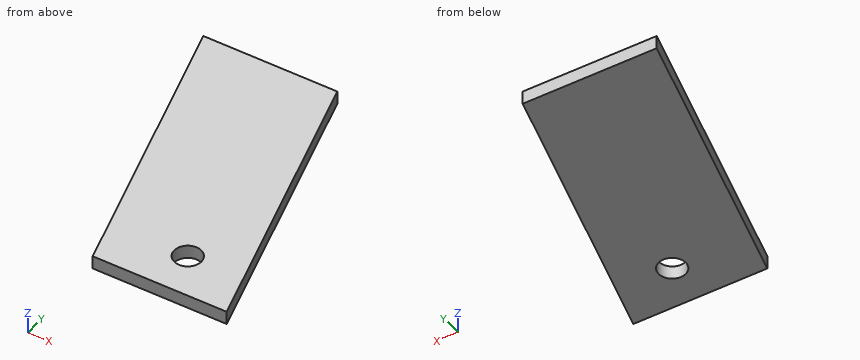
```python
from build123d import *

# Parameters (mm, degrees)
EXTRUDE_1_DEPTH     = 3
SKETCH_2_R          = 6.1
CUT_EXTRUDE_1_DEPTH = 15


with BuildPart() as part:
    # 草图1 → 凸台-拉伸1 (new, symmetric)
    with BuildSketch(Plane.XY):
        Polygon((-30, -36), (30, -36), (65, -167), (5, -167), align=None)
    extrude(amount=EXTRUDE_1_DEPTH, both=True)

    # 草图2 → 切除-拉伸1 (cut, symmetric)
    with BuildSketch(Plane.XY):
        with Locations(Location((35, -147.5, 0), (0, 0, 180))):
            Circle(SKETCH_2_R)
    extrude(amount=CUT_EXTRUDE_1_DEPTH, both=True, mode=Mode.SUBTRACT)


solid = part.part
```
The listing builds one solid part. Answer for the finished solid, in the listing's coordinates (mm). Give positions to 0.01 mm unless a question says otherwise; leave off trailing zeros. Order: outer loops, then holes, each group sorted by start corner. A loop starts at its lowest first (then second) coordinate and runs counter-clockwise, first axis right, second up.
1) Find section B-B on x = 35. Write down the section's boundary in (y, z).
Reported:
outline: (-167, -3) - (-153.6, -3) - (-153.6, 3) - (-167, 3) - close; (-141.4, -3) - (-54.71, -3) - (-54.71, 3) - (-141.4, 3) - close
2) Find section A-A on z = -0.6. Write down the section's boundary in (x, y), then the cut area to 3 significant figures.
Reported:
outline: (-30, -36) - (5, -167) - (65, -167) - (30, -36) - close; hole circle Ø12.2 at (35, -147.5)
area: 7,740 mm2
3) Consider line 1 along X through (y, z) = (-147.5, -0.4); line 2 along X through (y, z) = (-148.5, 1.55); line 3 along X through (y, z) = (-68.5, -1.55). Determine where each line is inside the solid, lowest interval first.
Reported:
line 1: x = -0.21 to 28.9, 41.1 to 59.79
line 2: x = 0.06 to 28.98, 41.02 to 60.06
line 3: x = -21.32 to 38.68
4) Given P1, Ø2, axis at y = -122, z = 0.5, coming from the +X side, flat-ended and moving along its own axis, determine where the tip first touches the part or whether it passes through.
Reported:
P1: stops at x = 53.24
5) Find section C-C on y = -147.5. Write down the section's boundary in (x, z), then the cut area to 3 significant figures.
Reported:
outline: (-0.21, -3) - (28.9, -3) - (28.9, 3) - (-0.21, 3) - close; (41.1, -3) - (59.79, -3) - (59.79, 3) - (41.1, 3) - close
area: 287 mm2
6) Find section D-D on y = -74.5. Write down the section's boundary in (x, z), then the cut area to 3 significant figures.
Reported:
outline: (-19.71, -3) - (40.29, -3) - (40.29, 3) - (-19.71, 3) - close
area: 360 mm2
